```python
from build123d import *

# Parameters (mm, degrees)
SKETCH1_R           = 25
BOSS_EXTRUDE1_DEPTH = 6.5
SKETCH2_R           = 21
BOSS_EXTRUDE3_DEPTH = 9
SKETCH5_R           = 15.5
CUT_EXTRUDE2_DEPTH  = 43
SKETCH6_R           = 17.5
CUT_EXTRUDE3_DEPTH  = 11
SKETCH7_R           = 17.5
SKETCH7_R_2         = 16.5
CUT_EXTRUDE4_DEPTH  = 0.5
CHAMFER1_SIZE       = 1


with BuildPart() as part:
    # Sketch1 → Boss-Extrude1 (new body)
    with BuildSketch(Plane.XY):
        with Locations(Location((0, 0, 0), (0, 0, 180))):
            Circle(SKETCH1_R)
    extrude(amount=BOSS_EXTRUDE1_DEPTH)

    # Sketch2 → Boss-Extrude3 (add)
    with BuildSketch(Plane.XY.offset(6.5)):
        Circle(SKETCH2_R)
    extrude(amount=BOSS_EXTRUDE3_DEPTH)

    # Sketch5 → Cut-Extrude2 (cut)
    with BuildSketch(Plane.XY.offset(15.5)):
        Circle(SKETCH5_R)
    extrude(amount=-CUT_EXTRUDE2_DEPTH, mode=Mode.SUBTRACT)

    # Sketch6 → Cut-Extrude3 (cut)
    with BuildSketch(Plane(origin=(0, 0, 0), x_dir=(-1, 0, 0), z_dir=(0, 0, -1))):
        Circle(SKETCH6_R)
    extrude(amount=-CUT_EXTRUDE3_DEPTH, mode=Mode.SUBTRACT)

    # Sketch7 → Cut-Extrude4 (cut)
    with BuildSketch(Plane(origin=(0, 0, 11), x_dir=(-1, 0, 0), z_dir=(0, 0, -1))):
        Circle(SKETCH7_R)
        Circle(SKETCH7_R_2, mode=Mode.SUBTRACT)
    extrude(amount=-CUT_EXTRUDE4_DEPTH, mode=Mode.SUBTRACT)

    # Chamfer1
    chamfer1_edges = [part.edges().sort_by_distance(p)[0] for p in [
        (25, 0, 0),
        (-21, 0, 15.5),
    ]]
    chamfer(chamfer1_edges, length=CHAMFER1_SIZE)


solid = part.part
```
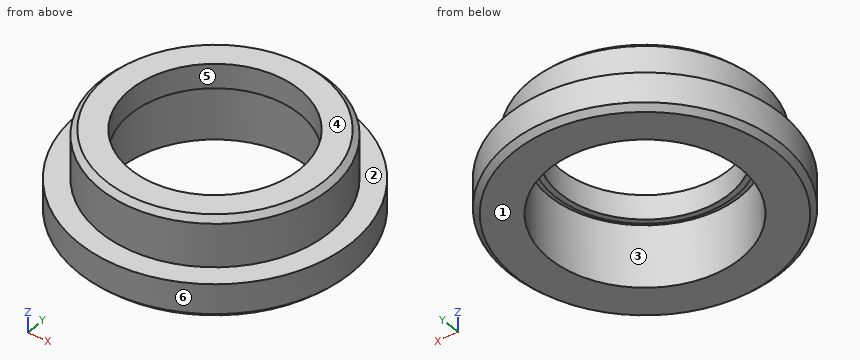
Source: CAD feature listing. Evaluate the final solid. Frame: model axes, mm. Face numbers are marked on the shaded views. A direction names the side the tool comes from. Give positions to 0.01 mm unless a question says otherwise; leave off trailing zeros. Write each loop counter-clockwise with the first axis right and the second up, starting at its lowest first coordinate (ties: lowest second). Pieces come first, ordered by that corner, then holes.
1. Pull-direction query (X, two-part tool) for the marked faces 4, 5 and 6; classes: +X half, -X half, draft (parallel to the pull), parting line (faces both ways), or undercut.
2. Section query C-C (z = 4). Return the cut outline in (x, y), then the cut area to 3 significant figures.
3. Access query for the marked faces 1, 2 and 3. Directions: +Z, -Z, +X, -X, +Y, -Y. A direction counts if a zero-diameter tool reaches every point of the face in a straight line with its end or side. Return the directions, or none.
4. Material intervals for line 1 along Y through (x, z) = (0, 12.65); line 2 along Y through (x, z) = (0, 2.5); line 3 along X through (y, z) = (4, 1), sorted ascending.
5. First-contact query: pin 1 (2 mm diameter, centred on y = -3, z = 3, fed in from +X); pin 2 (1 mm diameter, centred on y = 18, z = 5.5, fed in from +X); pin 3 (5 mm diameter, centred on y = -18.5, z = 3.5, fed in from +X); pin 4 (10 mm diameter, centred on x = -3.5, y = -5.5, fed in from -Z). Flat tips, straight axial feed; report the tip coordinate or a pass-through.
6. Section query A-A (y = 0). Return the cut outline in (x, z).
Output values:
1. face 4: draft
1. face 5: undercut
1. face 6: parting line
2. outline: circle Ø50 at (0, 0); hole circle Ø35 at (0, 0)
2. area: 1,000 mm2
3. face 1: -Z, +X, -X, +Y, -Y
3. face 2: +Z
3. face 3: -Z
4. line 1: y = -21 to -15.5, 15.5 to 21
4. line 2: y = -25 to -17.5, 17.5 to 25
4. line 3: x = -24.68 to -17.04, 17.04 to 24.68
5. pin 1: stops at x = 24.92
5. pin 2: stops at x = 17.85
5. pin 3: stops at x = 19.21
5. pin 4: passes through
6. outline: (-25, 1) - (-24, 0) - (-17.5, 0) - (-17.5, 11.5) - (-16.5, 11.5) - (-16.5, 11) - (-15.5, 11) - (-15.5, 15.5) - (-20, 15.5) - (-21, 14.5) - (-21, 6.5) - (-25, 6.5) - close; (15.5, 11) - (16.5, 11) - (16.5, 11.5) - (17.5, 11.5) - (17.5, 0) - (24, 0) - (25, 1) - (25, 6.5) - (21, 6.5) - (21, 14.5) - (20, 15.5) - (15.5, 15.5) - close
